Could you check a few things on this model? Use its own coordinates, in mm. A direction names the side the tool comes from. Round coordinates to 2 decimals unless told otherwise and drop trailing zeros. Write each loop counter-clockwise with the first axis right and the second up, starting at its lowest first coordinate (ties: lowest second). Pieces come first, ordered by that corner, then holes. Notation, with made-up numbers: (71, 27.5) -> (113, 27.5) arc R22 ccw to (113, 36.5) -> close; hole circle Ø2 at (-26.75, 30.25). An arc over 180 degrees is marked (long way). Answer in a Markdown table with one row per item.
from build123d import *

# Parameters (mm, degrees)
SKETCH_1_W             = 100
SKETCH_1_H             = 100
EXTRUDE_1_DEPTH        = 16
SKETCH_2_R             = 25
EXTRUDE_2_DEPTH        = 250
SKETCH_3_OUTSIDE_W     = 162.252
SKETCH_3_OUTSIDE_H     = 162.252
SKETCH_3_OUTSIDE_R     = 19.5
CUT_EXTRUDE_1_DEPTH    = 205
SKETCH_8_W             = 100
SKETCH_8_H             = 16
EXTRUDE_3_DEPTH        = 100
HOLE_WIZARD_M8_1_D     = 6.8
HOLE_WIZARD_M8_1_DEPTH = 19.75
HOLE_WIZARD_M8_1_TIP   = 2.042926105
HOLE_WIZARD_M10_1_D    = 11
CHAMFER_1_SIZE         = 10


with BuildPart() as part:
    # 草图1 → 凸台-拉伸1 (new body)
    with BuildSketch(Plane.XY):
        Rectangle(SKETCH_1_W, SKETCH_1_H)
    extrude(amount=EXTRUDE_1_DEPTH)

    # 草图2 → 凸台-拉伸2 (add)
    with BuildSketch(Plane.XY.offset(16)):
        Circle(SKETCH_2_R)
    extrude(amount=EXTRUDE_2_DEPTH)

    # 草图3 outside → 切除-拉伸1 (cut)
    with BuildSketch(Plane.XY.offset(266)):
        Rectangle(SKETCH_3_OUTSIDE_W, SKETCH_3_OUTSIDE_H)
        Circle(SKETCH_3_OUTSIDE_R, mode=Mode.SUBTRACT)
    extrude(amount=-CUT_EXTRUDE_1_DEPTH, mode=Mode.SUBTRACT)

    # 草图8 → 凸台-拉伸3 (add)
    with BuildSketch(Plane(origin=(0, 0, 0), x_dir=(-1, 0, 0), z_dir=(0, 0, -1))):
        with Locations((0, -42)):
            Rectangle(SKETCH_8_W, SKETCH_8_H)
    extrude(amount=EXTRUDE_3_DEPTH)

    # M8 螺纹孔1
    with Locations(Plane.XY.offset(266)):
        with Locations((0, 0)):
            Hole(HOLE_WIZARD_M8_1_D / 2, depth=HOLE_WIZARD_M8_1_DEPTH)
            with Locations((0, 0, -(HOLE_WIZARD_M8_1_DEPTH + HOLE_WIZARD_M8_1_TIP / 2))):  # 118° drill point
                Cone(0, HOLE_WIZARD_M8_1_D / 2, HOLE_WIZARD_M8_1_TIP, mode=Mode.SUBTRACT)

    # M10 间隙孔1 (through all)
    with Locations(Plane(origin=(0, -34, -18), x_dir=(1, 0, 0), z_dir=(0, 1, 0))):
        with Locations((-35, 67), (35, 67), (35, -3), (-35, -3)):
            Hole(HOLE_WIZARD_M10_1_D / 2)

    # 倒角1
    chamfer_1_edges = [part.edges().sort_by_distance(p)[0] for p in [
        (-50, -42, -100),
        (50, -42, -100),
        (-50, 50, 8),
        (50, 50, 8),
    ]]
    chamfer(chamfer_1_edges, length=CHAMFER_1_SIZE)


solid = part.part
1) For pin 1 (17.5 mm diameter, centred on x = 35, z = -15, fed in from -Y); pin 2 (17.5 mm diameter, centred on x = -35, z = -15, fed in from +Y); pin 3 (1.5 mm diameter, centred on x = 11, y = 11.5, fed in from -Z); pin 4 (3 mm diameter, centred on y = 16, z = 60.5, fed in from -X), each with a flat end and sliding along its axis, tell me the tip position at first contact or that it passes through.
Findings:
| item | result |
|---|---|
| pin 1 | stops at y = -50 |
| pin 2 | stops at y = -34 |
| pin 3 | stops at z = 0 |
| pin 4 | stops at x = -20.37 |
2) Imagine slicing it at D-D, the plane x = -8. Please give me the cut outline in (y, z), plus the area to 3 significant figures.
Findings:
| item | result |
|---|---|
| outline | (-50, -100) -> (-34, -100) -> (-34, 0) -> (50, 0) -> (50, 16) -> (23.69, 16) -> (23.69, 61) -> (17.78, 61) -> (17.78, 266) -> (-17.78, 266) -> (-17.78, 61) -> (-23.69, 61) -> (-23.69, 16) -> (-50, 16) -> close |
| area | 12,600 mm^2 |
3) Imagine slicing it at B-B, the plane x = 35. Please give me the cut outline in (y, z).
Findings:
| item | result |
|---|---|
| outline | (-50, -100) -> (-34, -100) -> (-34, -90.5) -> (-50, -90.5) -> close; (-50, -79.5) -> (-34, -79.5) -> (-34, -20.5) -> (-50, -20.5) -> close; (-50, -9.5) -> (-34, -9.5) -> (-34, 0) -> (50, 0) -> (50, 16) -> (-50, 16) -> close |
4) Imagine slicing it at A-A, the plane z = -15. Please give me the cut outline in (x, y).
Findings:
| item | result |
|---|---|
| outline | (-50, -50) -> (-40.5, -50) -> (-40.5, -34) -> (-50, -34) -> close; (-29.5, -50) -> (29.5, -50) -> (29.5, -34) -> (-29.5, -34) -> close; (40.5, -50) -> (50, -50) -> (50, -34) -> (40.5, -34) -> close |
5) Imagine slicing it at C-C, the plane y = -39. Please give me the cut outline in (x, z), plus the area to 3 significant figures.
Findings:
| item | result |
|---|---|
| outline | (-50, -90) -> (-40, -100) -> (40, -100) -> (50, -90) -> (50, 16) -> (-50, 16) -> close; hole circle Ø11 at (-35, -85); hole circle Ø11 at (-35, -15); hole circle Ø11 at (35, -85); hole circle Ø11 at (35, -15) |
| area | 11,100 mm^2 |
6) For faces 5 (the face through (1, -34, -49)), 6 (the face through (-45, 45, 8)), 7 (the face through (0.74, -3.32, 255.99)), which set-ups out of +Z, -Z, +X, -X, +Y, -Y let a thin tool reach every point of the face, with its end or its side?
Findings:
| item | result |
|---|---|
| face 5 | -Z, +X, -X, +Y |
| face 6 | +Z, -Z, -X, +Y |
| face 7 | +Z |
7) Please list where these lines run through material, in increasing order: line 1 (X direction, y = -44, z = -85); line 2 (Z direction, x = -35, y = -42); line 3 (Y direction, x = 0, z = 256).
Findings:
| item | result |
|---|---|
| line 1 | x = -50 to -40.5, -29.5 to 29.5, 40.5 to 50 |
| line 2 | z = -100 to -90.5, -79.5 to -20.5, -9.5 to 16 |
| line 3 | y = -19.5 to -3.4, 3.4 to 19.5 |
8) Thinking about a two-plate mould opening in X: for faces 1 (the face through (39.4, -42.1, -11.7)), 2 (the face through (-34.284, -42.112, -90.453)), 3 (the face through (50, -35, -25)), 4 (the face through (-50, -35, -25)), which applies, +X half, -X half, draft (parallel to the pull), parting line (faces both ways), or undercut?
Findings:
| item | result |
|---|---|
| face 1 | undercut |
| face 2 | undercut |
| face 3 | +X half |
| face 4 | -X half |
